CAD build for the part. Positions are in the model's coordinates, mm. A direction names the side the tool comes from. Coordinates: 2 decimals unless noted, no trailing zeros. Write each loop counter-clockwise with the first axis right and the second up, starting at its lowest first coordinate (ties: lowest second). Pieces come first, ordered by that corner, then holes. Notation, with made-up numbers: (-18, -15.75) - (0, -15.75) arc R17 cw to (0, 12.25) - close; hole circle Ø5 at (75, 65). An arc over 180 degrees is marked (long way). One line per question, with ' | ' between items. Start each with the question number.
1. Two-plate mould, pull along Y, no slides. Class faces 3 (the cylindrical face through (32.8, 247.1, -23)), 4 (the cylindrical face through (32.8, 247.1, 3)), 5 (the flat face through (37.4, 250, -10.1)), 6 (the flat face through (32, 149, 2)): +Y half, -Y half, draft (parallel to the pull), parting line (faces both ways), or undercut.
2. Band-saw the part on A-A, the plane y = 211. Write the cut outline in (x, z).
3. Which spindle directions (+Z, -Z, +X, -X, +Y, -Y) get a long thin tool onto all of the face, cutting with end or side? Do faces 1 (the flat face through (33, 149, -24)), 2 (the flat face through (32, 149, -22)). Say none if no direction does.
4. Probe line 1 (Y direction, x = 32, z = 3.15); line 2 (Z direction, x = 36.5, y = 213); line 3 (X direction, y = 232, z = -15.75). List the from-to ranges inside material, lowest first.
5. Band-saw the part on B-B, the plane z = -18.5. Write the cut outline in (x, y), then the cut area to 3 significant figures.
6. Flat gauge pin, fed straight in: P1, Ø6, axis at y = 158, z = -3, coming from the -X side. Where does the tip first touch, or does it go through?
from build123d import *

# Parameters (mm, degrees)
BOSS_EXTRUDE1_DEPTH     = 200
FILLET1_R               = 5
CUT_EXTRUDE1_DEPTH      = 255.356049663
CUT_EXTRUDE1_DEPTH_BACK = 255.356049663
SKETCH3_R               = 2.5
CUT_EXTRUDE2_DEPTH      = 255.356049663
CUT_EXTRUDE2_DEPTH_BACK = 255.356049663
SKETCH9_R               = 2.5


with BuildPart() as part:
    # Sketch2 → Boss-Extrude1 (new body)
    with BuildSketch(Plane(origin=(0, 50, 0), x_dir=(1, 0, 0), z_dir=(0, 1, 0))):
        Polygon((27, 22), (37, 22), (37, -2), (27, -2), (27, -4), (39, -4), (39, 24), (27, 24), align=None)
    extrude(amount=BOSS_EXTRUDE1_DEPTH)

    # Fillet1
    fillet1_edges = [part.edges().sort_by_distance(p)[0] for p in [
        (27, 50, 3),
        (27, 50, -23),
    ]]
    fillet(fillet1_edges, radius=FILLET1_R)

    # Sketch3 → Cut-Extrude1 (cut, two sides: drawn at the far end of the back side and taken through both)
    with BuildSketch(Plane(origin=(0, 0, 2), x_dir=(-1, 0, 0), z_dir=(0, 0, -1)).offset(-CUT_EXTRUDE1_DEPTH_BACK)):
        with Locations((-32, 55)):
            Circle(SKETCH3_R)
    extrude(amount=CUT_EXTRUDE1_DEPTH + CUT_EXTRUDE1_DEPTH_BACK, mode=Mode.SUBTRACT)

    # Sketch9 → Cut-Extrude2 (cut, two sides: drawn at the far end of the back side and taken through both)
    with BuildSketch(Plane(origin=(0, 0, -22), x_dir=(-1, 0, 0), z_dir=(0, 0, -1)).offset(-CUT_EXTRUDE2_DEPTH_BACK)):
        with Locations(Location((-32, 244.730145932, 0), (0, 0, 90))):
            Circle(SKETCH9_R)
    extrude(amount=CUT_EXTRUDE2_DEPTH + CUT_EXTRUDE2_DEPTH_BACK, mode=Mode.SUBTRACT)


solid = part.part
Filled in:
1) face 3: undercut | face 4: undercut | face 5: +Y half | face 6: draft
2) outline: (27, -24) - (39, -24) - (39, 4) - (27, 4) - (27, 2) - (37, 2) - (37, -22) - (27, -22) - close
3) face 1: -Z, +X, -X, +Y, -Y | face 2: -X, +Y, -Y
4) line 1: y = 50 to 52.5, 57.5 to 242.23, 247.23 to 250 | line 2: z = -24 to -22, 2 to 4 | line 3: x = 37 to 39
5) outline: (37, 50) - (39, 50) - (39, 250) - (37, 250) - close | area: 400 mm²
6) P1: stops at x = 37
